Answer from the drawing. Dimensions are ordinates in mm from the lowest x, y and z of the part. Give positions to 0.01 mm unless a question says otherwise; leave off trailing zeros. Write each loop counter-clockwise with the first axis right and the second up, starting at its lowest first coordinate (ties: lowest second). Pieces come first, ordered by that corner, then holes.
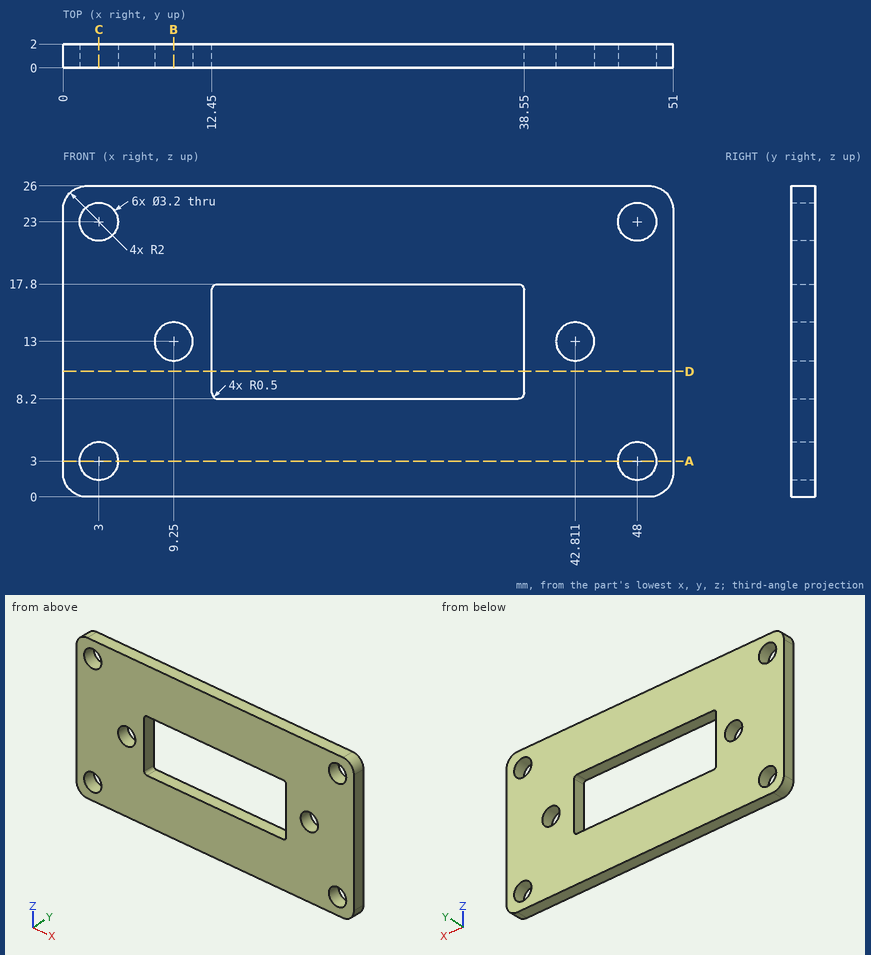
Item 1: A cutting plane is placed at B-B, the plane x = 9.25. Give the vertices of the cut face in (y, z), plus the area to 3 significant figures.
Conclusion:
outline: (0, 0) - (2, 0) - (2, 11.4) - (0, 11.4) - close; (0, 14.6) - (2, 14.6) - (2, 26) - (0, 26) - close
area: 45.6 mm2
Item 2: A cutting plane is placed at C-C, the plane x = 3. Give the vertices of the cut face in (y, z), plus the area to 3 significant figures.
Conclusion:
outline: (0, 0) - (2, 0) - (2, 1.4) - (0, 1.4) - close; (0, 4.6) - (2, 4.6) - (2, 21.4) - (0, 21.4) - close; (0, 24.6) - (2, 24.6) - (2, 26) - (0, 26) - close
area: 39.2 mm2
Item 3: Each of these flat-tipped pins is pushed along its axis until it touches: P1, Ø10, axis at x = 37.5, z = 11.5, coming from the +Y side; P2, Ø2.5, axis at x = 9.25, z = 13, coming from the +Y side. Where does it stop, or does it pass through?
Conclusion:
P1: stops at y = 2
P2: passes through
Item 4: Consider probe 1 along X at (y, z) = (1.1, 23); probe 2 along Z at (x, y) = (22, 1.55); probe 3 along X at (y, z) = (0.6, 10.25). Determine where each line is inside the solid, lowest interval first.
Conclusion:
probe 1: x = 0 to 1.4, 4.6 to 46.4, 49.6 to 51
probe 2: z = 0 to 8.2, 17.8 to 26
probe 3: x = 0 to 12.45, 38.55 to 51
Item 5: A cutting plane is placed at D-D, the plane z = 10.5. Give the vertices of the cut face in (x, y), plus the area to 3 significant figures.
Conclusion:
outline: (0, 0) - (12.45, 0) - (12.45, 2) - (0, 2) - close; (38.55, 0) - (51, 0) - (51, 2) - (38.55, 2) - close
area: 49.8 mm2
Item 6: A cutting plane is placed at A-A, the plane z = 3. Give the vertices of the cut face in (x, y).
Conclusion:
outline: (0, 0) - (1.4, 0) - (1.4, 2) - (0, 2) - close; (4.6, 0) - (46.4, 0) - (46.4, 2) - (4.6, 2) - close; (49.6, 0) - (51, 0) - (51, 2) - (49.6, 2) - close
